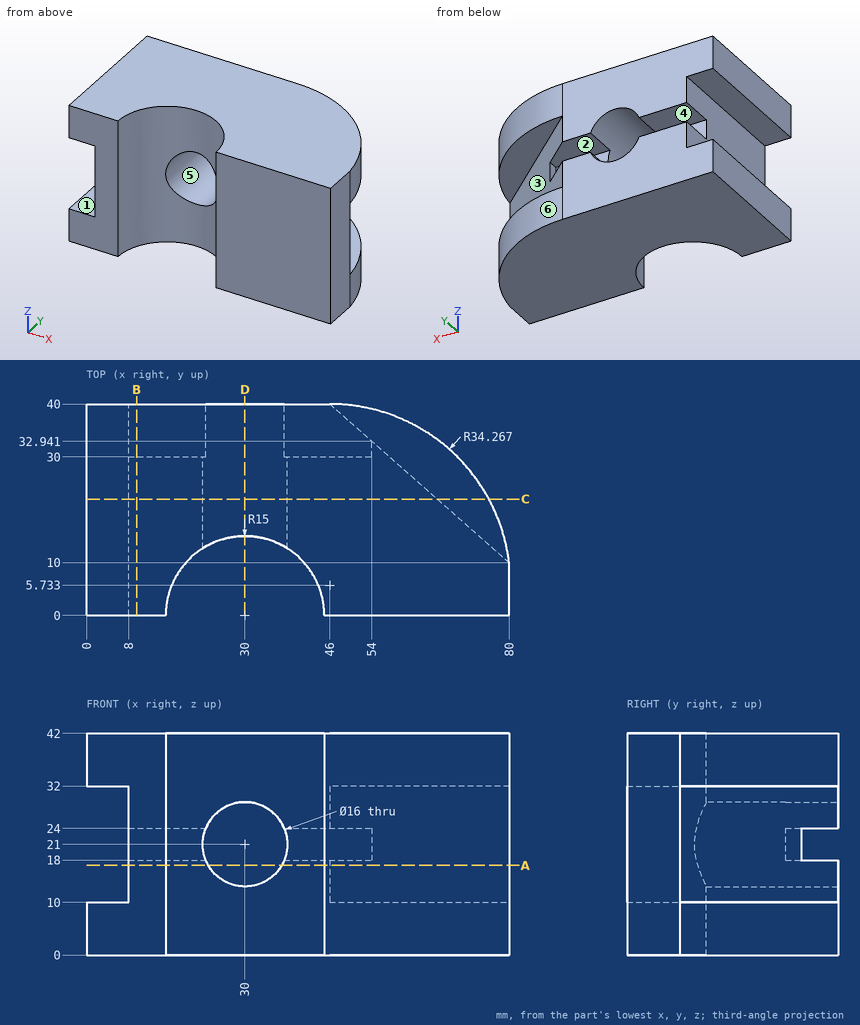
Could you check a few things on this drawing? It's one solid part, dimensions in mm from its lowest x, y, z. A direction names the side the tool comes from. Round coordinates to 2 decimals unless told otherwise and drop trailing zeros. Order: outer loops, then holes, each group sorted by start corner. A loop starts at its lowest first (then second) coordinate and runs counter-clockwise, first axis right, second up.
Q1. Please list where these lines run through material, in increasing order: probe 1 along Z at (x, y) = (53.5, 32); probe 2 along Z at (x, y) = (26.5, 16.5) (1 decimal); probe 3 along X at (y, z) = (23.5, 21).
Geometry says:
probe 1: z = 0 to 18, 24 to 42
probe 2: z = 0 to 13.8, 28.2 to 42
probe 3: x = 8 to 22, 38 to 64.7
Q2. Imagine slicing it at A-A, the plane z = 17. List the corners of the cut face in (x, y) for me.
Geometry says:
outline: (8, 0) - (15, 0) arc R15 cw to (23.07, 13.3) - (23.07, 40) - (8, 40) - close; (36.93, 13.3) arc R15 cw to (45, 0) - (80, 0) - (80, 10) - (46, 40) - (36.93, 40) - close
Q3. Imagine slicing it at B-B, the plane x = 9.5. List the corners of the cut face in (y, z) for me.
Geometry says:
outline: (0, 0) - (40, 0) - (40, 18) - (30, 18) - (30, 24) - (40, 24) - (40, 42) - (0, 42) - close
Q4. I'm going to push flat-ended pins straight in: P1, Ø3, axis at y = 30.5, z = 35.5, coming from the +X side; P2, Ø5, axis at y = 32, z = 27, coming from the -X side; P3, Ø3, axis at x = 17, z = 20, coming from the +Y side. Where does each tip first touch, or does it pass through?
Geometry says:
P1: stops at x = 71.16
P2: stops at x = 8
P3: stops at y = 30
Q5. Thinking about a two-plate mould opening in X: for the marked faces 4, 5 and 6, which applies, released by +X, released by -X, zero draft, split by the parting line, or undercut?
Geometry says:
face 4: zero draft
face 5: undercut
face 6: released by +X
Q6. Imagine slicing it at D-D, the plane x = 30. List the corners of the cut face in (y, z) for me, then the cut area to 3 significant figures.
Geometry says:
outline: (15, 0) - (40, 0) - (40, 13) - (15, 13) - close; (15, 29) - (40, 29) - (40, 42) - (15, 42) - close
area: 650 mm2
Q7. Imagine slicing it at C-C, the plane y = 22. List the corners of the cut face in (x, z) for me.
Geometry says:
outline: (0, 0) - (76.16, 0) - (76.16, 10) - (66.4, 10) - (66.4, 32) - (76.16, 32) - (76.16, 42) - (0, 42) - (0, 32) - (8, 32) - (8, 10) - (0, 10) - close; hole circle Ø16 at (30, 21)
Q8. Which directions (+Z, -Z, +X, -X, +Y, -Y) give clear straight access to the entire face, cutting with the end or side of a thin tool? Please do the marked faces 1, 2 and 3.
Geometry says:
face 1: -X, +Y, -Y
face 2: -X, +Y
face 3: +X, +Y
